Input: part model. Units: mm. Frame: model coordinates. Round coordinates to 2 decimals unless told otherwise and drop trailing zeros. Order: outer loops, then holes, each group sorted by start corner. A loop starts at its lowest first (then second) coordinate and runs counter-clockwise, first axis right, second up.
Item 1: Cut plane D-D on y = 4.25. Output: boundary loops of the cut face in (x, z).
Item 2: Cut plane C-C on z = 0.4. Output: boundary loops of the cut face in (x, y), then the cut area to 3 significant figures.
Item 3: Cut plane A-A on y = -2. Output: boundary loops of the cut face in (x, z).
Item 4: Line query: L1, parallel to X at y = 0, z = 0.6; L2, parallel to X at y = 1, z = 0.1. Output: solid intervals per line, ascending.
Item 5: Cut plane B-B on x = 3. Output: boundary loops of the cut face in (y, z), then the cut area to 3 significant figures.
Item 6: Mould query, pull axis X, two halves, no side actions, for faces 1 (the flat face through (1.449, -4.69, 0.493)), 2 (the flat face through (3.92, 1.42, 1)). Classes: released by +X, released by -X, zero draft, split by the parting line, or undercut.
```python
from build123d import *

# Parameters (mm, degrees)
SKETCH1_R           = 6
SKETCH1_R_2         = 4
BOSS_EXTRUDE1_DEPTH = 1
CUT_EXTRUDE1_DEPTH  = 9.544003745


with BuildPart() as part:
    # Sketch1 → Boss-Extrude1 (new body)
    with BuildSketch(Plane.XY):
        Circle(SKETCH1_R)
        Circle(SKETCH1_R_2, mode=Mode.SUBTRACT)
    extrude(amount=BOSS_EXTRUDE1_DEPTH)

    # Sketch2 → Cut-Extrude1 (cut, through all)
    with BuildSketch(Plane(origin=(0, 0, 0), x_dir=(1, 0, 0), z_dir=(0, 1, 0))):
        Polygon((0, 0), (0.95899064, 0), (1.953022833, -1), (0.994032193, -1), align=None)
    extrude(amount=-CUT_EXTRUDE1_DEPTH, mode=Mode.SUBTRACT)


solid = part.part
```
From the geometry:
1. outline: (-4.24, 0) - (4.24, 0) - (4.24, 1) - (-4.24, 1) - close
2. outline: (0.4, -5.99) - (0.4, -3.98) arc R4 cw (long way) to (1.36, -3.76) - (1.36, -5.84) arc R6 ccw (long way) to start
2. area: 60.9 mm2
3. outline: (-5.66, 0) - (-3.46, 0) - (-3.46, 1) - (-5.66, 1) - close; (3.46, 0) - (5.66, 0) - (5.66, 1) - (3.46, 1) - close
4. L1: x = -6 to -4, 4 to 6
4. L2: x = -5.92 to -3.87, 3.87 to 5.92
5. outline: (-5.2, 0) - (-2.65, 0) - (-2.65, 1) - (-5.2, 1) - close; (2.65, 0) - (5.2, 0) - (5.2, 1) - (2.65, 1) - close
5. area: 5.10 mm2
6. face 1: undercut
6. face 2: zero draft
